```python
from build123d import *

# Parameters (mm, degrees)
SKETCH2_R          = 7.5
CUT_EXTRUDE1_DEPTH = 31
SKETCH3_W          = 40.68
SKETCH3_H          = 6
CUT_EXTRUDE2_DEPTH = 8.5
CIRPATTERN1_COUNT  = 4
CHAMFER1_SIZE      = 0.5
CHAMFER2_SIZE      = 0.5


with BuildPart() as part:
    # Sketch1 → Revolve1 (revolve)
    with BuildSketch(Plane.XY, mode=Mode.PRIVATE) as revolve1_sk:
        Polygon((0, 0), (-14, 0), (-14, 3.5), (-16, 3.5), (-16, 8), (-10, 14), (0, 14), align=None)
    revolve(revolve1_sk.sketch.rotate(Axis((0, 0, 0), (0, 1, 0)), 270), axis=Axis((0, 0, 0), (0, 1, 0)))

    # Sketch2 → Cut-Extrude1 (cut)
    with BuildSketch(Plane(origin=(0, 14, 0), x_dir=(1, 0, 0), z_dir=(0, 1, 0))):
        with Locations(Location((0, 0, 0), (0, 0, 270))):
            Circle(SKETCH2_R)
    extrude(amount=-CUT_EXTRUDE1_DEPTH, mode=Mode.SUBTRACT)

    # Sketch3 → Cut-Extrude2 (cut)
    with BuildSketch(Plane(origin=(0, 14, 0), x_dir=(1, 0, 0), z_dir=(0, 1, 0))):
        Rectangle(SKETCH3_W, SKETCH3_H)
    cut_extrude2 = extrude(amount=-CUT_EXTRUDE2_DEPTH, mode=Mode.SUBTRACT)

    # CirPattern1: Cut-Extrude2 ×4 about axis
    cirpattern1_axis = Axis((0, -17, 0), (0, 1, 0))
    for i in range(1, CIRPATTERN1_COUNT):
        add(cut_extrude2.rotate(cirpattern1_axis, i * 360 / CIRPATTERN1_COUNT), mode=Mode.SUBTRACT)

    # Chamfer1
    chamfer1_edges = [part.edges().sort_by_distance(p)[0] for p in [
        (0, 0, 14),
    ]]
    chamfer(chamfer1_edges, length=CHAMFER1_SIZE)

    # Chamfer2
    chamfer2_edges = [part.edges().sort_by_distance(p)[0] for p in [
        (0, 0, -7.5),
    ]]
    chamfer(chamfer2_edges, length=CHAMFER2_SIZE)


solid = part.part
```
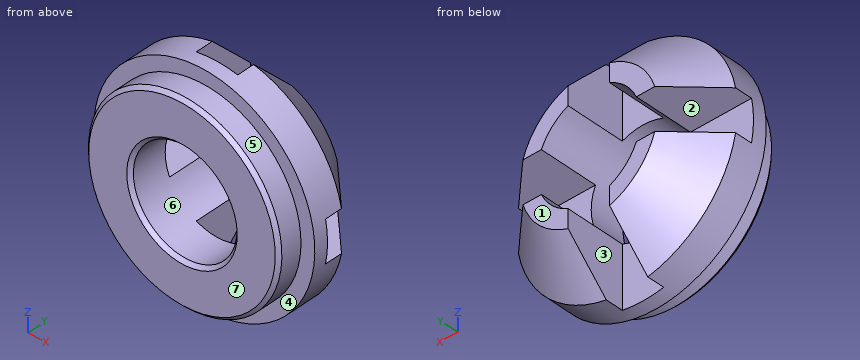
Source: CAD feature listing. Evaluate the final solid. Frame: model axes, mm. Face numbers are marked on the shaded views. A direction names the side the tool comes from. Give positions to 0.01 mm unless a question says otherwise; leave off trailing zeros. Order: outer loops, then holes, each group sorted by start corner. A loop starts at its lowest first (then second) coordinate and runs counter-clockwise, first axis right, second up.
(1) Section query B-B (x = 0). Return the cut outline in (y, z).
(2) Contact query for flat-ended pins moving along their axis: P1, Ø2.5, axis at y = 10.5, z = 9.5, coming from the -X side; P2, Ø5, axis at x = -12, y = 10, coming from the -Z side; P3, Ø3, axis at x = 13, z = -0.5, coming from the +Y side; P4, Ø8, axis at x = 5, z = 10, coming from the +Y side. Output: stop coordinate, or through.
(3) Material intervals for line 1 along Y through (x, z) = (11, 2.5); line 2 along X through (y, z) = (4.5, 0.5); line 3 along Z through (x, y) = (-8, 6.25), sorted ascending.
(4) Section query D-D (y = 5). Return the cut outline in (x, z).
(5) Pull-direction query (X, two-part tool) for the marked faces 5, 6 and 7; classes: +X half, -X half, draft (parallel to the pull), parting line (faces both ways), or undercut.
(6) Access query for the marked faces 1, 2, 3 and 4. Directions: +Z, -Z, +X, -X, +Y, -Y. A direction counts if a zero-diameter tool reaches every point of the face in a straight line with its end or side. Return the directions, or none.
(7) Section query C-C (y = 11.5). Return the cut outline in (x, z), plus the area to 3 significant figures.
(8) Section query A-A (z = 0). Return the cut outline in (x, y).
Outcome:
1. outline: (0, -13.5) - (0.5, -14) - (3.5, -14) - (3.5, -16) - (5.5, -16) - (5.5, -7.5) - (0.5, -7.5) - (0, -8) - close; (0, 8) - (0.5, 7.5) - (5.5, 7.5) - (5.5, 16) - (3.5, 16) - (3.5, 14) - (0.5, 14) - (0, 13.5) - close
2. P1: stops at x = -11.57
2. P2: stops at z = -12.07
2. P3: stops at y = 5.5
2. P4: stops at y = 14
3. line 1: y = 0 to 5.5
3. line 2: x = -15.99 to -7.48, 7.48 to 15.99
3. line 3: z = -13.86 to -3, 3 to 13.86
4. outline: circle Ø32 at (0, 0); hole circle Ø15 at (0, 0)
5. face 5: parting line
5. face 6: undercut
5. face 7: draft
6. face 1: +Z, -Z, +X, -X, +Y
6. face 2: +X, -X, +Y
6. face 3: +Z, -Z, +Y
6. face 4: -Y
7. outline: (-12.13, -3) arc R12.5 ccw to (-3, -12.13) - (-3, -6.87) arc R7.5 cw to (-6.87, -3) - close; (-12.13, 3) - (-6.87, 3) arc R7.5 cw to (-3, 6.87) - (-3, 12.13) arc R12.5 ccw to start; (3, -12.13) arc R12.5 ccw to (12.13, -3) - (6.87, -3) arc R7.5 cw to (3, -6.87) - close; (3, 6.87) arc R7.5 cw to (6.87, 3) - (12.13, 3) arc R12.5 ccw to (3, 12.13) - close
7. area: 192 mm2
8. outline: (-16, 3.5) - (-14, 3.5) - (-14, 0.5) - (-13.5, 0) - (-8, 0) - (-7.5, 0.5) - (-7.5, 5.5) - (-16, 5.5) - close; (7.5, 0.5) - (8, 0) - (13.5, 0) - (14, 0.5) - (14, 3.5) - (16, 3.5) - (16, 5.5) - (7.5, 5.5) - close
